Part print with two shaded views. Sizes in mm from the minimum x, y, z corner. Give positions to 0.01 mm unless a question says otherwise; leave off trailing zeros. Order: outer loops, then holes, each group sorted by start corner. A loop starts at its lowest first (then second) coordinate and runs counter-clockwise, first axis right, second up. Notation, with made-up numbers: M -32,34.5 L 27,34.5 A13 ccw 27,56.5 Z; hole C -39,4.5 d5. An arc over 180 degrees is marked long. Answer as CSV lines item,"result".
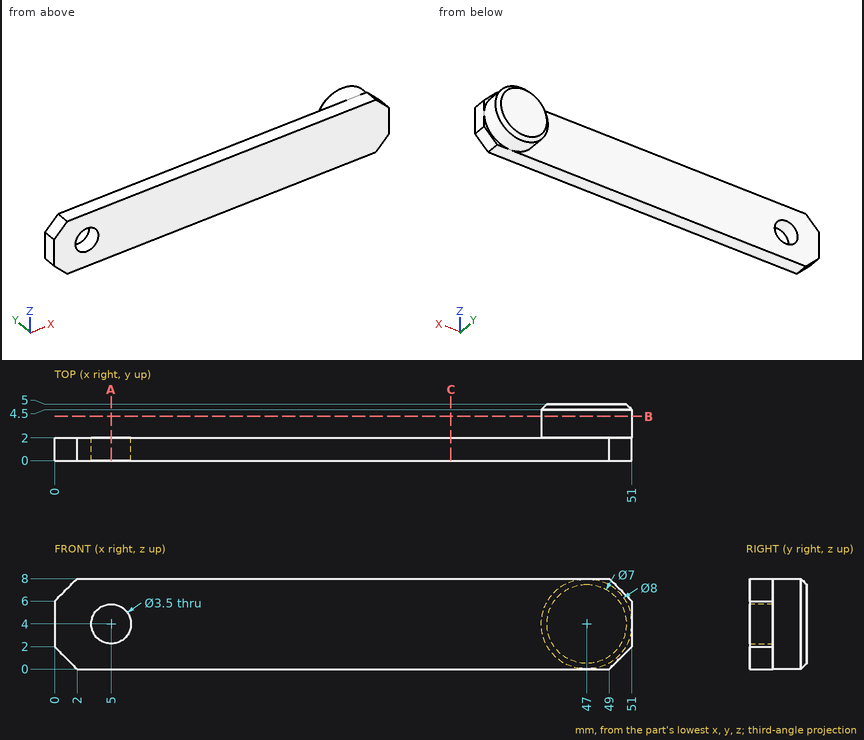
Item 1: Drop flat-ended pins along their axis: pin 1 (1 mm diameter, centred on x = 17, z = 3, fed in from +Y); pin 2 (1 mm diameter, centred on x = 8, y = 3.5, fed in from -Z). Give the stop position or say it passes through.
Geometry says:
pin 1,"stops at y = 2"
pin 2,"passes through"
Item 2: Band-saw the part on C-C (x = 35). Give the cut face in (y, z), and give its area (3 significant figures).
Geometry says:
outline,"M 0,0 L 2,0 L 2,8 L 0,8 Z"
area,"16.0 mm2"
Item 3: Probe line 1 along Y through (x, z) = (34.5, 0.75); line 2 along X through (y, z) = (3.2, 1.5); line 3 along Z through (x, y) = (44, 4.2). List the from-to ranges inside material, lowest first. Write a range as from..to.
Geometry says:
line 1,"y = 0..2"
line 2,"x = 43.88..50.12"
line 3,"z = 1.35..6.65"
Item 4: Band-saw the part on A-A (x = 5). Give the cut face in (y, z).
Geometry says:
outline,"M 0,0 L 2,0 L 2,2.25 L 0,2.25 Z; M 0,5.75 L 2,5.75 L 2,8 L 0,8 Z"
Item 5: Band-saw the part on B-B (y = 3.9). Give the cut face in (x, z), and give its area (3 significant figures).
Geometry says:
outline,"C 47,4 d8"
area,"50.3 mm2"
